The listing builds one solid part. Answer for the finished solid, in the listing's coordinates (mm). A direction names the side the tool comes from. Round coordinates to 2 decimals unless told otherwise and drop trailing zeros. Order: outer loops, then holes, each group sorted by start corner. A loop starts at its lowest first (then second) coordinate and runs counter-clockwise, first axis right, second up. Notation, with made-up numbers: (31.25, 42) -> (75.25, 42) arc R17 ccw to (75.25, 53) -> close; hole circle Ø9 at (35.5, -3). An arc over 180 degrees is marked (long way). Return JSON: item names as keys, results as strings. Group by question number.
(1) The part is cut by section C-C (z = -2). Determine the outline of the cut face in (x, y), plus the area to 3 significant figures.
(2) Which of the six approach directions +Z, -Z, +X, -X, +Y, -Y give full straight-line access (tool end or side, diameter ignored) to faces 1 (the face through (-5.1, -1, 2.2)), 2 (the face through (-1, 3, 0))?
(3) The part is cut by section A-A (y = 0). Determine the outline of the cut face in (x, z).
(4) The part is cut by section B-B (x = 0). Determine the outline of the cut face in (y, z).
(5) Consider line 1 (Z direction, x = 4.5, y = -1.25); line 2 (Y direction, x = 0, z = -9.5); line 3 (Y direction, x = 3.5, z = 1.25). Determine where each line is inside the solid, lowest interval first. Write a range as [from, to].
(6) Each of these flat-tipped pins is pushed along its axis until it touches: pin 1 (5 mm diameter, centred on x = -1, z = -14, fed in from +Y); pin 2 (6 mm diameter, centred on x = 1.5, z = -6, fed in from -Y); pin 3 (1.5 mm diameter, centred on y = 1, z = -17.5, fed in from -X). Where does it stop, or does it pass through?
(7) The part is cut by section D-D (x = 3.5). Determine the outline of the cut face in (y, z), plus the area to 3 significant figures.
from build123d import *

# Parameters (mm, degrees)
SKETCH1_R           = 6
BOSS_EXTRUDE1_DEPTH = 4.5
SKETCH2_OUTSIDE_W   = 17.512
SKETCH2_OUTSIDE_H   = 17.512
CUT_EXTRUDE1_DEPTH  = 4.5
SKETCH3_R           = 3
BOSS_EXTRUDE2_DEPTH = 20
CHAMFER2_SIZE       = 1


with BuildPart() as part:
    # Sketch1 → Boss-Extrude1 (new body)
    with BuildSketch(Plane.XY):
        Circle(SKETCH1_R)
    extrude(amount=BOSS_EXTRUDE1_DEPTH)

    # Sketch2 outside → Cut-Extrude1 (cut)
    with BuildSketch(Plane(origin=(0, 0, 0), x_dir=(-1, 0, 0), z_dir=(0, 0, -1))):
        Rectangle(SKETCH2_OUTSIDE_W, SKETCH2_OUTSIDE_H)
        Polygon((4.581142128, -3.874678929), (5.646141448, 2.030045997), (1.06499932, 5.904724926), (-4.581142128, 3.874678929), (-5.646141448, -2.030045997), (-1.06499932, -5.904724926), align=None, mode=Mode.SUBTRACT)
    extrude(amount=-CUT_EXTRUDE1_DEPTH, mode=Mode.SUBTRACT)

    # Sketch3 → Boss-Extrude2 (add)
    with BuildSketch(Plane(origin=(0, 0, 0), x_dir=(-1, 0, 0), z_dir=(0, 0, -1))):
        Circle(SKETCH3_R)
    extrude(amount=BOSS_EXTRUDE2_DEPTH)

    # Chamfer2
    chamfer2_edges = [part.edges().sort_by_distance(p)[0] for p in [
        (3, 0, -20),
    ]]
    chamfer(chamfer2_edges, length=CHAMFER2_SIZE)


solid = part.part
Answer below:
{
 "1": {"outline": "circle Ø6 at (0, 0)", "area": "28.3 mm²"},
 "2": {"face 1": "+Z, -Z, -X, -Y", "face 2": "-Z"},
 "3": {"outline": "(-5.28, 0) -> (-3, 0) -> (-3, -19) -> (-2, -20) -> (2, -20) -> (3, -19) -> (3, 0) -> (5.28, 0) -> (5.28, 4.5) -> (-5.28, 4.5) -> close"},
 "4": {"outline": "(-5.52, 0) -> (-3, 0) -> (-3, -19) -> (-2, -20) -> (2, -20) -> (3, -19) -> (3, 0) -> (5.52, 0) -> (5.52, 4.5) -> (-5.52, 4.5) -> close"},
 "5": {"line 1": "z = [0, 4.5]", "line 2": "y = [-3, 3]", "line 3": "y = [-3.85, 4.26]"},
 "6": {"pin 1": "stops at y = 3", "pin 2": "stops at y = -3", "pin 3": "stops at x = -2.99"},
 "7": {"outline": "(-3.85, 0) -> (4.26, 0) -> (4.26, 4.5) -> (-3.85, 4.5) -> close", "area": "36.5 mm²"}
}
